Input: part model. Units: mm. Frame: model coordinates. Give positions to 0.01 mm unless a question says otherwise; leave off trailing zeros. Loops run counter-clockwise (first coordinate to the right, second up) from the corner with the lowest first, then second, coordinate; pieces in that order, holes last. Notation, with made-up numbers: (-3.5, 12.25) -> (21.5, 12.25) arc R16 ccw to (21.5, 27.25) -> close; hole circle Ø10 at (60, 22). An arc over 180 degrees is marked (long way). Use CSV: the item, a comma, the result in double quotes.
```python
from build123d import *


with BuildPart() as part:
    # Sketch 181 → 旋转1 (revolve)
    with BuildSketch(Plane.XY, mode=Mode.PRIVATE) as revolve_1_sk:
        Polygon((-30, 40.77255102), (-29.2, 40), (29.2, 40), (30, 40.77255102), (30, 52.5), (22.5, 52.5), (22.5, 47.3), (20.5, 47.3), (20.5, 47.5), (-29.2, 47.5), (-30, 46.7), align=None)
    revolve(revolve_1_sk.sketch.rotate(Axis((-30, 0, 0), (1, 0, 0)), 90), axis=Axis((-30, 0, 0), (1, 0, 0)))


solid = part.part
```
1) Section query A-A (y = 0). Return loops of the section in (x, z), then the cut area to 3 significant figures.
From the geometry:
outline,"(-30, -46.7) -> (-29.2, -47.5) -> (20.5, -47.5) -> (20.5, -47.3) -> (22.5, -47.3) -> (22.5, -52.5) -> (30, -52.5) -> (30, -40.77) -> (29.2, -40) -> (-29.2, -40) -> (-30, -40.77) -> close; (-30, 40.77) -> (-29.2, 40) -> (29.2, 40) -> (30, 40.77) -> (30, 52.5) -> (22.5, 52.5) -> (22.5, 47.3) -> (20.5, 47.3) -> (20.5, 47.5) -> (-29.2, 47.5) -> (-30, 46.7) -> close"
area,"972 mm^2"
2) Mould query, pull axis X, two halves, no side actions, for faces 1 (the flat face through (-30, 41, 0)), 2 (the cylindrical face through (-4.7, 46.37, -10.3)), 3 (the cylindrical face through (21.486, 46.175, -10.254)). Classes: pulls with the +X half, pulls with the -X half, needs draft (parallel to the pull), parting line crosses it, or undercut.
From the geometry:
face 1,"pulls with the -X half"
face 2,"needs draft"
face 3,"undercut"
3) Contact query for flat-ended pins moving along their axis: pin 1 (1 mm diameter, centred on x = -23.5, z = 17, fed in from -Y); pin 2 (1.5 mm diameter, centred on x = -18.5, y = -33.5, fed in from -Z); pin 3 (4 mm diameter, centred on x = 4.5, y = -18, fed in from +Z). Output: stop coordinate, or through.
From the geometry:
pin 1,"stops at y = -44.54"
pin 2,"stops at z = -34.4"
pin 3,"stops at z = 44.72"
4) Section query C-C (x = -6.5). Return loops of the section in (y, z).
From the geometry:
outline,"circle Ø95 at (0, 0); hole circle Ø80 at (0, 0)"
5) Ray query, line 1 (Y direction, x = 5, z = 0); line 2 (X direction, y = -41, z = 27); line 3 (Z direction, x = 25, y = -13). Return the intervals inside material, ascending.
From the geometry:
line 1,"y = -47.5 to -40, 40 to 47.5"
line 2,"x = 22.5 to 30"
line 3,"z = -50.87 to -37.83, 37.83 to 50.87"
